```python
from build123d import *

# Parameters (mm, degrees)
SKETCH2_W                                            = 20
SKETCH2_H                                            = 31
BOSS_EXTRUDE1_DEPTH                                  = 6
SKETCH3_W                                            = 1.4
SKETCH3_H                                            = 31
BOSS_EXTRUDE2_DEPTH                                  = 2
SKETCH4_W                                            = 2
SKETCH4_H                                            = 17.5
CUT_EXTRUDE1_DEPTH                                   = 27.537709019
CBORE_FOR_M2_HEXAGON_SOCKET_HEAD_CAP_SCR_D           = 2.4
CBORE_FOR_M2_HEXAGON_SOCKET_HEAD_CAP_SCR_DEPTH       = 10.1
CBORE_FOR_M2_HEXAGON_SOCKET_HEAD_CAP_SCR_CBORE_D     = 4.3
CBORE_FOR_M2_HEXAGON_SOCKET_HEAD_CAP_SCR_CBORE_DEPTH = 2.3
CBORE_FOR_M2_HEXAGON_SOCKET_HEAD_CAP_SCR_TIP         = 0.721032743
M3_TAPPED_HOLE1_D                                    = 2.5
M3_TAPPED_HOLE1_DEPTH                                = 7.5
M3_TAPPED_HOLE1_TIP                                  = 0.751075774
CHAMFER1_SIZE                                        = 1


with BuildPart() as part:
    # Sketch2 → Boss-Extrude1 (new body)
    with BuildSketch(Plane(origin=(0, 0, 0), x_dir=(0, 0, -1), z_dir=(1, 0, 0))):
        Rectangle(SKETCH2_W, SKETCH2_H)
    extrude(amount=BOSS_EXTRUDE1_DEPTH)

    # Sketch3 → Boss-Extrude2 (add)
    with BuildSketch(Plane(origin=(6, 0, 0), x_dir=(0, 0, -1), z_dir=(1, 0, 0))):
        with Locations((-9.3, 0)):
            Rectangle(SKETCH3_W, SKETCH3_H)
        with Locations((9.3, 0)):
            Rectangle(SKETCH3_W, SKETCH3_H)
    extrude(amount=BOSS_EXTRUDE2_DEPTH)

    # Sketch4 → Cut-Extrude1 (cut, through all)
    with BuildSketch(Plane.XY.offset(10)):
        with Locations((7, -6.75)):
            Rectangle(SKETCH4_W, SKETCH4_H)
    extrude(amount=-CUT_EXTRUDE1_DEPTH, mode=Mode.SUBTRACT)

    # CBORE for M2 Hexagon socket head cap screws1
    with Locations(Plane.ZY):
        with Locations((6, 12.5), (-6, 12.5), (-6, 4.5), (6, 4.5)):
            CounterBoreHole(CBORE_FOR_M2_HEXAGON_SOCKET_HEAD_CAP_SCR_D / 2, CBORE_FOR_M2_HEXAGON_SOCKET_HEAD_CAP_SCR_CBORE_D / 2, CBORE_FOR_M2_HEXAGON_SOCKET_HEAD_CAP_SCR_CBORE_DEPTH, depth=CBORE_FOR_M2_HEXAGON_SOCKET_HEAD_CAP_SCR_DEPTH)
            with Locations((0, 0, -(CBORE_FOR_M2_HEXAGON_SOCKET_HEAD_CAP_SCR_DEPTH + CBORE_FOR_M2_HEXAGON_SOCKET_HEAD_CAP_SCR_TIP / 2))):  # 118° drill point
                Cone(0, CBORE_FOR_M2_HEXAGON_SOCKET_HEAD_CAP_SCR_D / 2, CBORE_FOR_M2_HEXAGON_SOCKET_HEAD_CAP_SCR_TIP, mode=Mode.SUBTRACT)

    # M3 Tapped Hole1
    with Locations(Plane(origin=(0, -15.5, 0), x_dir=(-1, 0, 0), z_dir=(0, -1, 0))):
        with Locations((-3, 5), (-3, -5)):
            Hole(M3_TAPPED_HOLE1_D / 2, depth=M3_TAPPED_HOLE1_DEPTH)
            with Locations((0, 0, -(M3_TAPPED_HOLE1_DEPTH + M3_TAPPED_HOLE1_TIP / 2))):  # 118° drill point
                Cone(0, M3_TAPPED_HOLE1_D / 2, M3_TAPPED_HOLE1_TIP, mode=Mode.SUBTRACT)

    # Chamfer1
    chamfer1_edges = [part.edges().sort_by_distance(p)[0] for p in [
        (3, -15.5, -10),
        (3, -15.5, 10),
    ]]
    chamfer(chamfer1_edges, length=CHAMFER1_SIZE)


solid = part.part
```
Input: part model. Units: mm. Frame: model coordinates. A direction names the side the tool comes from. Coordinates: 2 decimals unless noted, no trailing zeros. Write each loop counter-clockwise with the first axis right and the second up, starting at its lowest first coordinate (ties: lowest second). Pieces come first, ordered by that corner, then holes. Notation, with made-up numbers: M 37,25.25 L 75,25.25 A5 ccw 75,34.25 Z; hole C 42,1.5 d9. An arc over 180 degrees is marked long. Use one line per item in the form item = value.
Q1. Section B-B (y = 12.5). Return loops of the section in (x, z).
Answer below:
outline = M 0,-10 L 8,-10 L 8,-8.6 L 6,-8.6 L 6,-7.2 L 2.3,-7.2 L 2.3,-8.15 L 0,-8.15 Z; M 0,-3.85 L 2.3,-3.85 L 2.3,-4.8 L 6,-4.8 L 6,4.8 L 2.3,4.8 L 2.3,3.85 L 0,3.85 Z; M 0,8.15 L 2.3,8.15 L 2.3,7.2 L 6,7.2 L 6,8.6 L 8,8.6 L 8,10 L 0,10 Z
Q2. Section C-C (x = 5.25). Return loops of the section in (y, z), plus the area to 3 significant figures.
Answer below:
outline = M -15.5,-9 L -14.5,-10 L 15.5,-10 L 15.5,10 L -14.5,10 L -15.5,9 Z; hole C 4.5,-6 d2.4; hole C 4.5,6 d2.4; hole C 12.5,-6 d2.4; hole C 12.5,6 d2.4
area = 601 mm²
Q3. Section D-D (y = -11). Return loops of the section in (x, z), plus the area to 3 significant figures.
Answer below:
outline = M 0,-10 L 6,-10 L 6,10 L 0,10 Z; hole C 3,-5 d2.5; hole C 3,5 d2.5
area = 110 mm²
Q4. Draft query along Z for faces 6 (the face through (3, -15, -9.5)), 7 (the face through (0, 0, 0)), 8 (the face through (4.18, 5.69, 6.16)). Return one class per face: released by +Z, released by -Z, zero draft, split by the parting line, or undercut.
Answer below:
face_6 = released by -Z
face_7 = zero draft
face_8 = undercut
Q5. Set-up query: faces 1 (the face through (3.577, -11.698, 6.109)), 2 (the face through (7, 9, -8.6)), 3 (the face through (7, 2, -9)), 4 (the face through (4, 0, -10)), 5 (the face through (1.134, 11.192, -7.706)). Return all of +Z, -Z, +X, -X, +Y, -Y with unobstructed straight access to the full face (end or side cutting, diameter ignored); none if empty.
Answer below:
face_1 = -Y
face_2 = +X, +Y, -Y
face_3 = +Z, -Z, +X, -Y
face_4 = -Z, +X, -X, +Y, -Y
face_5 = -X
Q6. Section A-A (x = 7.25). Return loops of the section in (y, z), plus the area to 3 significant figures.
Answer below:
outline = M 2,-10 L 15.5,-10 L 15.5,-8.6 L 2,-8.6 Z; M 2,8.6 L 15.5,8.6 L 15.5,10 L 2,10 Z
area = 37.8 mm²
Q7. Material intervals for probe 1 along Y at (x, z) = (1.85, 6); probe 2 along X at (y, z) = (-13.5, 5); probe 3 along Y at (x, z) = (2, 4.75), sorted ascending. Write a range as from..to.
Answer below:
probe_1 = -15.5..2.35, 6.65..10.35, 14.65..15.5
probe_2 = 0..1.75, 4.25..6
probe_3 = -7.87..2.75, 6.25..10.75, 14.25..15.5
Q8. First-contact query: pin 1 (1.5 mm diameter, centred on x = 7, z = 9.5, fed in from -Y); pin 2 (3.5 mm diameter, centred on y = 4.5, z = 6, fed in from +X); pin 3 (2 mm diameter, centred on y = 12.5, z = -6.5, fed in from -X). Flat tips, straight axial feed; report the tip coordinate or a pass-through.
Answer below:
pin_1 = 2
pin_2 = 6
pin_3 = 2.3
